Could you check a few things on this model? Use its own coordinates, in mm. A direction names the side the tool comes from. Give positions to 0.01 mm unless a question says otherwise; leave off trailing zeros. Order: outer loops, then holes, each group sorted by start corner. A loop starts at its lowest first (then second) coordinate and runs counter-clockwise, first axis right, second up. Notation, with made-up numbers: M 55,29 L 112,29 A17 ccw 112,38 Z; hole C 19,0.25 d3. An arc over 180 degrees is marked long. Answer in a Markdown table with one row per item. Add a question column.
```python
from build123d import *

# Parameters (mm, degrees)
SKETCH1_W           = 240
SKETCH1_H           = 240
BOSS_EXTRUDE1_DEPTH = 11
SKETCH2_R           = 109.5
SKETCH2_R_2         = 103.5
CUT_EXTRUDE1_DEPTH  = 0.5
SKETCH3_R           = 7
CUT_EXTRUDE2_DEPTH  = 59
CHAMFER1_SIZE       = 3


with BuildPart() as part:
    # Sketch1 → Boss-Extrude1 (new body)
    with BuildSketch(Plane.XY):
        Rectangle(SKETCH1_W, SKETCH1_H)
    extrude(amount=BOSS_EXTRUDE1_DEPTH)

    # Sketch2 → Cut-Extrude1 (cut)
    with BuildSketch(Plane.XY.offset(11)):
        Circle(SKETCH2_R)
        Circle(SKETCH2_R_2, mode=Mode.SUBTRACT)
    extrude(amount=-CUT_EXTRUDE1_DEPTH, mode=Mode.SUBTRACT)

    # Sketch3 → Cut-Extrude2 (cut)
    with BuildSketch(Plane.XY.offset(11)):
        with Locations((-95, 95)):
            Circle(SKETCH3_R)
        with Locations((95, 95)):
            Circle(SKETCH3_R)
        with Locations((95, -95)):
            Circle(SKETCH3_R)
        with Locations((-95, -95)):
            Circle(SKETCH3_R)
    extrude(amount=-CUT_EXTRUDE2_DEPTH, mode=Mode.SUBTRACT)

    # Chamfer1
    chamfer1_edges = [part.edges().sort_by_distance(p)[0] for p in [
        (-120, 120, 5.5),
        (120, 120, 5.5),
        (120, -120, 5.5),
        (-120, -120, 5.5),
    ]]
    chamfer(chamfer1_edges, length=CHAMFER1_SIZE)


solid = part.part
```
1. For faces 1 (the flat face through (-1, 1, 11)), 2 (the cylindrical face through (-23.737, -106.896, 10.754)), which set-ups out of +Z, -Z, +X, -X, +Y, -Y let a thin tool reach every point of the face, with its end or its side?
2. If I drill on line 1 along Y through (x, z) = (95, 5.5); line 2 along X through (y, z) = (-99, 7.75), over which ranges is the centre line in solid material (lowest first)? Write a range as [from, to].
3. Suppose I cut it at A-A on y = 95. List the corners of the cut face in (x, z) for me, plus the area to 3 significant figures.
4. Thinking about a two-plate mould opening in X: for faces 3 (the cylindrical face through (98.72, 31.09, 10.75)), 4 (the cylindrical face through (-100.16, 99.73, 5.58)), 5 (the flat face through (-2, -120, 5)), 6 (the flat face through (120, -2, 5)), which applies, pulls with the +X half, pulls with the -X half, needs draft (parallel to the pull), parting line crosses it, or undercut?
5. Will this pin go through, and if not, where does the flat tip stop? P1, Ø8.5, axis at x = -95, y = -95, coming from the -Z side.
Findings below:
| question | item | result |
|---|---|---|
| 1 | face 1 | +Z, +X, -X, +Y, -Y |
| 1 | face 2 | +Z |
| 2 | line 1 | [-120, -102], [-88, 88], [102, 120] |
| 2 | line 2 | [-120, -100.74], [-89.26, 89.26], [100.74, 120] |
| 3 | outline | M -120,0 L -102,0 L -102,11 L -120,11 Z; M -88,0 L 88,0 L 88,11 L 54.45,11 L 54.45,10.5 L 41.08,10.5 L 41.08,11 L -41.08,11 L -41.08,10.5 L -54.45,10.5 L -54.45,11 L -88,11 Z; M 102,0 L 120,0 L 120,11 L 102,11 Z |
| 3 | area | 2,320 mm2 |
| 4 | face 3 | undercut |
| 4 | face 4 | undercut |
| 4 | face 5 | needs draft |
| 4 | face 6 | pulls with the +X half |
| 5 | P1 | through |
